The drawing under review shows one solid part. Ordinate dimensions are in mm from its lowest x, y, z. A direction names the side the tool comes from. Round coordinates to 2 decimals unless told otherwise and drop trailing zeros. Order: outer loops, then holes, each group sorted by start corner. A loop starts at its lowest first (then second) coordinate and runs counter-clockwise, first axis right, second up. Notation, with made-up numbers: M -32,67.5 L 17,67.5 A24 cw 17,89.5 Z; hole C 14,54.25 d2. An arc over 180 degrees is marked long. Write item = value, one per line. Start each with the question number.
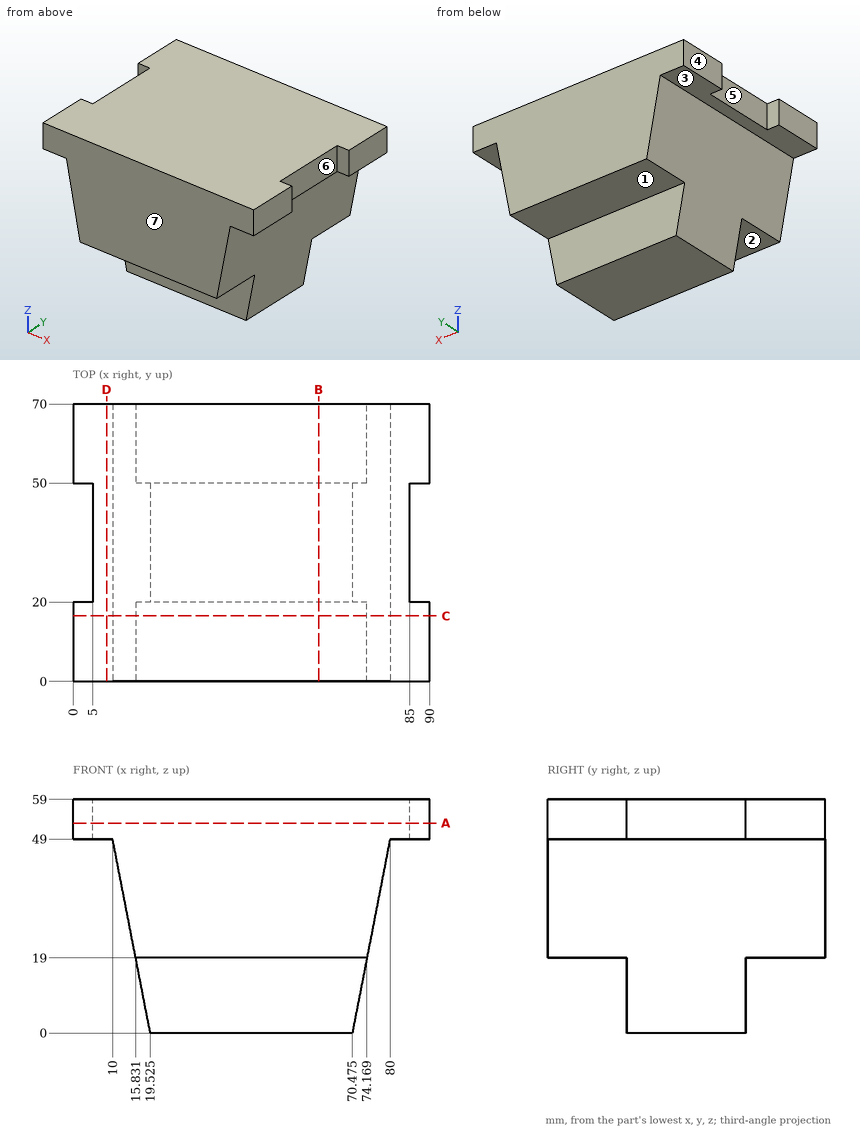
(1) Draft analysis for pull direction Y (two halves, no side actions). For the marked faces 4, 5, 6 and 7, state which applies: pulls with the +Y half, pulls with the -Y half, needs draft (parallel to the pull), parting line crosses it, or undercut.
(2) Consider section C-C, the plane y = 16.5. Write out the cut boundary in (x, z), then the cut area to 4 significant figures.
(3) Consider section A-A, the plane z = 53. Write out the cut boundary in (x, y), then the cut area to 3 significant figures.
(4) For line 1 along Z through (x, y) = (41, 55); line 2 along Z through (x, y) = (6, 55.5); line 3 along Y through (x, z) = (60.5, 16), list the stretches that pass through material, from the lowest coordinate up. Write a range as [from, to].
(5) Consider section D-D, the plane x = 8.5. Write out the cut boundary in (y, z), then the cut area to 3 significant figures.
(6) Consider section B-B, the plane x = 62. Write out the cut boundary in (y, z), then the cut area to 3 significant figures.
(7) Insertion check: pin 1 (3 mm diameter, centred on x = 87, y = 18, fed in from -Z); pin 2 (9.5 mm diameter, centred on x = 54, z = 9.5, fed in from -Y); pin 3 (10 mm diameter, centred on x = 50, y = 59.5, fed in from -Z). Each pin has a flat end and moves straight along its axis. Give the tip position at first contact, or say it passes through.
(8) For the marked faces 1, 2 and 3, list the 3-axis set-ups (+Z, -Z, +X, -X, +Y, -Y) from which the entire face can be reached by the end or side of a thin tool; tool diameter is ignored.
Completed:
q1.face_4 = needs draft
q1.face_5 = undercut
q1.face_6 = undercut
q1.face_7 = pulls with the -Y half
q2.outline = M 0,49 L 10,49 L 15.83,19 L 74.17,19 L 80,49 L 90,49 L 90,59 L 0,59 Z
q2.area = 2,825 mm2
q3.outline = M 0,0 L 90,0 L 90,20 L 85,20 L 85,50 L 90,50 L 90,70 L 0,70 L 0,50 L 5,50 L 5,20 L 0,20 Z
q3.area = 6,000 mm2
q4.line_1 = [19, 59]
q4.line_2 = [49, 59]
q4.line_3 = [20, 50]
q5.outline = M 0,49 L 70,49 L 70,59 L 0,59 Z
q5.area = 700 mm2
q6.outline = M 0,19 L 20,19 L 20,0 L 50,0 L 50,19 L 70,19 L 70,59 L 0,59 Z
q6.area = 3,370 mm2
q7.pin_1 = 49
q7.pin_2 = 20
q7.pin_3 = 19
q8.face_1 = -Z, +X, -X, +Y
q8.face_2 = -Z, +X, -X, -Y
q8.face_3 = -Z, -X, +Y, -Y
